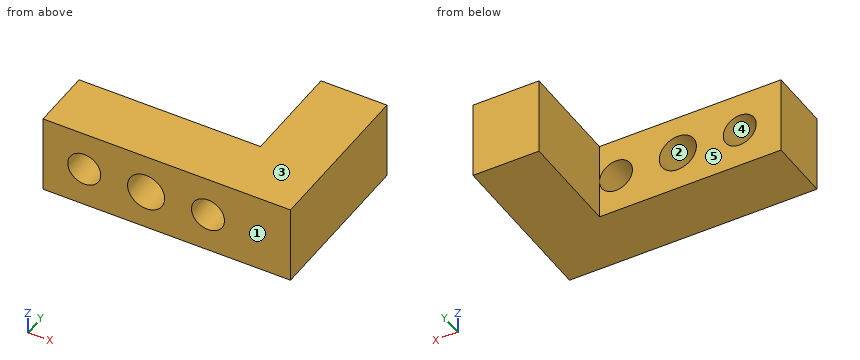
from build123d import *

# Parameters (mm, degrees)
BOSS_EXTRUDE1_DEPTH = 19
SKETCH2_R           = 4
SKETCH2_R_2         = 4.5
CUT_EXTRUDE1_DEPTH  = 15


with BuildPart() as part:
    # Sketch1 → Boss-Extrude1 (new body)
    with BuildSketch(Plane.XY):
        Polygon((0, 0), (60, 0), (60, 40.20000018), (44, 40.20000018), (44, 15), (0, 15), align=None)
    extrude(amount=BOSS_EXTRUDE1_DEPTH)

    # Sketch2 → Cut-Extrude1 (cut)
    with BuildSketch(Plane(origin=(0, 0, 0), x_dir=(-1, 0, 0), z_dir=(0, -1, 0))):
        with Locations(Location((-10, -9.5, 0), (0, 0, 90))):
            Circle(SKETCH2_R)
        with Locations(Location((-25, -9.5, 0), (0, 0, 90))):
            Circle(SKETCH2_R_2)
        with Locations(Location((-40, -9.5, 0), (0, 0, 90))):
            Circle(SKETCH2_R)
    extrude(amount=-CUT_EXTRUDE1_DEPTH, mode=Mode.SUBTRACT)


solid = part.part
Can you work these out from the model? Positions are in its coordinate system, mm. Face numbers are marked on the shaded views. A direction names the side the tool comes from. Round coordinates to 2 decimals unless told otherwise and drop trailing zeros. Write each loop counter-clockwise with the first axis right and the second up, starting at its lowest first coordinate (ties: lowest second). Pieces come first, ordered by that corner, then holes. Notation, with made-up numbers: (-7, 89.25) -> (30, 89.25) arc R26 cw to (30, 124.25) -> close; hole circle Ø10 at (9.25, 76). An arc over 180 degrees is marked (long way). Use one line per item in the form item = value. Start each with the question number.
Q1. Imagine slicing it at D-D (z = 17.5). Please give me the cut outline in (x, y), then the cut area to 3 significant figures.
Q2. We'd pull the mould along Z, two halves only. Please class the marked faces 1, 2 and 3: +Z half, -Z half, draft (parallel to the pull), parting line (faces both ways), or undercut.
Q3. Imagine slicing it at B-B (y = 12). Please give me the cut outline in (x, z), then the cut area to 3 significant figures.
Q4. Imagine slicing it at C-C (z = 6.5). Please give me the cut outline in (x, y), then the cut area to 3 significant figures.
Q5. I'm going to push flat-ended pins straight in: P1, Ø3, axis at x = 24, z = 14.5, coming from the +Y side; P2, Ø1.5, axis at y = 31.5, z = 12.5, coming from the -X side. Where does each tip first touch, or does it pass through?
Q6. Which directions (+Z, -Z, +X, -X, +Y, -Y) give clear straight access to the entire face, cutting with the end or side of a thin tool? Please do the marked faces 4 and 5.
Q7. Imagine slicing it at A-A (x = 10). Please give me the cut outline in (y, z), then the cut area to 3 significant figures.
Q8. If I drill on probe 1 along X at (y, z) = (11.5, 9.5); probe 2 along X at (y, z) = (3.5, 11); probe 3 along Z at (x, y) = (40, 9.5), over which ranges is the centre line in solid material (lowest first)? Write a range as [from, to].
Worked out:
q1.outline = (0, 0) -> (60, 0) -> (60, 40.2) -> (44, 40.2) -> (44, 15) -> (0, 15) -> close
q1.area = 1,300 mm^2
q2.face_1 = draft
q2.face_2 = undercut
q2.face_3 = +Z half
q3.outline = (0, 0) -> (60, 0) -> (60, 19) -> (0, 19) -> close; hole circle Ø8 at (10, 9.5); hole circle Ø9 at (25, 9.5); hole circle Ø8 at (40, 9.5)
q3.area = 976 mm^2
q4.outline = (0, 0) -> (7.35, 0) -> (7.35, 15) -> (0, 15) -> close; (12.65, 0) -> (21.65, 0) -> (21.65, 15) -> (12.65, 15) -> close; (28.35, 0) -> (37.35, 0) -> (37.35, 15) -> (28.35, 15) -> close; (42.65, 0) -> (60, 0) -> (60, 40.2) -> (44, 40.2) -> (44, 15) -> (42.65, 15) -> close
q4.area = 1,040 mm^2
q5.P1 = 15
q5.P2 = 44
q6.face_4 = +Y, -Y
q6.face_5 = +Z, -Z, -X, +Y
q7.outline = (0, 0) -> (15, 0) -> (15, 5.5) -> (0, 5.5) -> close; (0, 13.5) -> (15, 13.5) -> (15, 19) -> (0, 19) -> close
q7.area = 165 mm^2
q8.probe_1 = [0, 6], [14, 20.5], [29.5, 36], [44, 60]
q8.probe_2 = [0, 6.29], [13.71, 20.76], [29.24, 36.29], [43.71, 60]
q8.probe_3 = [0, 5.5], [13.5, 19]
